```python
from build123d import *

# Parameters (mm, degrees)
SKETCH1_W           = 1200
SKETCH1_H           = 80
SKETCH1_R           = 12.5
SKETCH1_R_2         = 3
BOSS_EXTRUDE1_DEPTH = 2


with BuildPart() as part:
    # Sketch1 → Boss-Extrude1 (new body)
    with BuildSketch(Plane(origin=(0, 0, 0), x_dir=(1, 0, 0), z_dir=(0, 1, 0))):
        Rectangle(SKETCH1_W, SKETCH1_H)
        with Locations(Location((-400, 0, 0), (0, 0, 270))):
            Circle(SKETCH1_R, mode=Mode.SUBTRACT)
        with Locations(Location((400, 0, 0), (0, 0, 270))):
            Circle(SKETCH1_R, mode=Mode.SUBTRACT)
        with Locations(Location((-577.5, 20, 0), (0, 0, 270))):
            Circle(SKETCH1_R_2, mode=Mode.SUBTRACT)
        with Locations(Location((577.5, 20, 0), (0, 0, 270))):
            Circle(SKETCH1_R_2, mode=Mode.SUBTRACT)
        with Locations(Location((-577.5, -20, 0), (0, 0, 270))):
            Circle(SKETCH1_R_2, mode=Mode.SUBTRACT)
        with Locations(Location((577.5, -20, 0), (0, 0, 270))):
            Circle(SKETCH1_R_2, mode=Mode.SUBTRACT)
        with Locations(Location((0, 0, 0), (0, 0, 270))):
            Circle(SKETCH1_R, mode=Mode.SUBTRACT)
    extrude(amount=BOSS_EXTRUDE1_DEPTH)


solid = part.part
```
Geometry check sheet. Reference: the model listing, model coordinates, mm. Give positions to 0.01 mm unless a question says otherwise; leave off trailing zeros. Loops run counter-clockwise (first coordinate to the right, second up) from the corner with the lowest first, then second, coordinate; pieces in that order, holes last. Notation, with made-up numbers: M 88,-10.5 L 127,-10.5 A31 cw 127,26.5 Z; hole C -33.5,-30.75 d8. An arc over 180 degrees is marked long. Write item = value, one per line.
(1) Gauge pin test, flat end, axial feed: pin 1 Ø5 at (x, z) = (577.5, -20) entering from +Y (3 decimals). Record the tip position at first contact, or that the pin passes through.
Answer below:
pin_1 = through
(2) Sectioned sample at A-A, the plane z = 0. Record the cut outline in (x, y), plus the area to 3 significant figures.
Answer below:
outline = M -600,0 L -412.5,0 L -412.5,2 L -600,2 Z; M -387.5,0 L -12.5,0 L -12.5,2 L -387.5,2 Z; M 12.5,0 L 387.5,0 L 387.5,2 L 12.5,2 Z; M 412.5,0 L 600,0 L 600,2 L 412.5,2 Z
area = 2,250 mm2
(3) Material ranges on line 1 (X direction, y = 0.85, z = 20); line 2 (Z direction, x = -577.5, y = 0.7); line 3 (X direction, y = 0.7, z = -0.5), recorded low to high. Write a range as [from, to].
Answer below:
line_1 = [-600, -580.5], [-574.5, 574.5], [580.5, 600]
line_2 = [-40, -23], [-17, 17], [23, 40]
line_3 = [-600, -412.49], [-387.51, -12.49], [12.49, 387.51], [412.49, 600]
(4) Sectioned sample at C-C, the plane y = 0.4. Record the cut outline in (x, z), plus the area to 3 significant figures.
Answer below:
outline = M -600,-40 L 600,-40 L 600,40 L -600,40 Z; hole C -577.5,-20 d6; hole C -577.5,20 d6; hole C -400,0 d25; hole C 0,0 d25; hole C 400,0 d25; hole C 577.5,-20 d6; hole C 577.5,20 d6
area = 94,400 mm2
(5) Sectioned sample at B-B, the plane x = -400. Record the cut outline in (y, z), plus the area to 3 significant figures.
Answer below:
outline = M 0,-40 L 2,-40 L 2,-12.5 L 0,-12.5 Z; M 0,12.5 L 2,12.5 L 2,40 L 0,40 Z
area = 110 mm2
(6) Release check for a two-part mould opening along X. For faces 1 (the face through (388.91, 0.99, 5.77)), 2 (the face through (-411.09, 0.99, 5.77)), 3 (the face through (-8, 0, -18)) record: released by +X, released by -X, zero draft, split by the parting line, or undercut.
Answer below:
face_1 = undercut
face_2 = undercut
face_3 = zero draft
